The listing builds one solid part. Answer for the finished solid, in the listing's coordinates (mm). Face numbers are marked on the shaded views. A direction names the side the tool comes from. Give positions to 0.01 mm unless a question says otherwise; leave off trailing zeros. Loops run counter-clockwise (first coordinate to the right, second up) from the corner with the lowest first, then second, coordinate; pieces in that order, holes last. Notation, with made-up numbers: (33, 57) - (48, 57) arc R23 ccw to (48, 65) - close; hole circle Ø11 at (-17, -3). An arc over 180 degrees is marked (long way). Write item = value, one per line. Start each with the question number.
1) The part is cut by section C-C on y = 8. Write down the section's boundary in (x, z).
2) The part is cut by section A-A on z = 8. Write down the section's boundary in (x, y), plus the area to 3 significant figures.
3) The part is cut by section B-B on y = -45. Write down the section's boundary in (x, z), plus the area to 3 significant figures.
4) Which of the six approach directions +Z, -Z, +X, -X, +Y, -Y give full straight-line access (tool end or side, diameter ignored) to the marked faces 1, 2, 3 and 4?
5) The part is cut by section D-D on x = -38. Write down the section's boundary in (y, z), plus the area to 3 significant figures.
6) Consider probe 1 along Z at (x, y) = (-15.5, -44.5); probe 2 along Z at (x, y) = (45, 41); probe 3 along Y at (x, z) = (-13.5, 32). Determine where each line is inside the solid, lowest interval first.
7) The mould has two halves that part along X. Classify the marked faces 5, 6 and 7: +X half, -X half, draft (parallel to the pull), parting line (faces both ways), or undercut.
8) Flat-ended cylindrical pins translate along their axes: P1, Ø20, axis at x = 0.5, y = -57, coming from the -Z side; P2, Ø10, axis at x = 31.5, z = 48, coming from the +Y side; P3, Ø21, axis at x = -64.95, y = 37.5, coming from the -Z side; P4, Ø19, axis at x = 45, y = -44.5, coming from the +Z side. Find the tip coordinate at first contact, or state that the pin passes through.
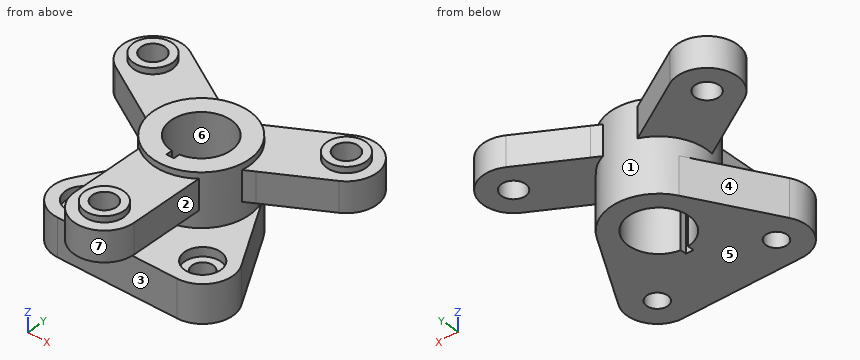
from build123d import *

# Parameters (mm, degrees)
BASE_BLOCK_DEPTH            = 25
HUB_SKETCH_64_R             = 32
HUB_64_DEPTH                = 31
THREE_START                 = -20
THREE_ARMS_120DEG_DEPTH     = 20
HUB_COLLAR_SKETCH_64_R      = 32
HUB_COLLAR_64X4_DEPTH       = 4
BOLT_BOSSES_SKETCH_3X_13_R  = 13
BOLT_BOSSES_3X_13_DEPTH     = 4
BOLT_HOLES_SKETCH_3X_8_R    = 8
BOLT_HOLES_3X_8_DEPTH       = 25
KEYED_BORE_24_DEPTH         = 80
COUNTERBORE_SKETCH_2X_12_R  = 12
COUNTERBORES_2X_12X6_DEPTH  = 6
THROUGH_HOLES_SKETCH_2X_7_R = 7
THROUGH_HOLES_2X_7_DEPTH    = 50


with BuildPart() as part:
    # Base Block Sketch → Base Block (new body)
    with BuildSketch(Plane.XY):
        with BuildLine():
            Line((-57.296551724, -34.95862069), (-27.674482759, 16.066206897))
            ThreePointArc((-27.674482759, 16.066206897), (0, 32), (27.674482759, 16.066206897))
            Line((27.674482759, 16.066206897), (57.296551724, -34.95862069))
            ThreePointArc((57.296551724, -34.95862069), (57.332449137, -54.979288897), (40, -65))
            Line((40, -65), (-40, -65))
            ThreePointArc((-40, -65), (-57.332449137, -54.979288897), (-57.296551724, -34.95862069))
        make_face()
    extrude(amount=BASE_BLOCK_DEPTH)

    # Hub Sketch _64 → Hub _64 (add)
    with BuildSketch(Plane.XY.offset(25)):
        with Locations(Location((0, 0, 0), (0, 0, 149.863023681))):
            Circle(HUB_SKETCH_64_R)
    extrude(amount=HUB_64_DEPTH)

    # Three Arms Sketch → Three Arms 120deg (add)
    with BuildSketch(Plane.XY.offset(56).offset(THREE_START)):
        with BuildLine():
            Line((-20, -75), (-20, -24.979991994))
            ThreePointArc((-20, -24.979991994), (0, -32), (20, -24.979991994))
            Line((20, -24.979991994), (20, -75))
            ThreePointArc((20, -75), (0, -95), (-20, -75))
        make_face()
        with BuildLine():
            Line((-11.633307653, 29.810504072), (-54.951905284, 54.820508076))
            ThreePointArc((-54.951905284, 54.820508076), (-82.27241336, 47.5), (-74.951905284, 20.179491924))
            Line((-74.951905284, 20.179491924), (-31.633307653, -4.830512079))
            ThreePointArc((-31.633307653, -4.830512079), (-27.712812921, 16), (-11.633307653, 29.810504072))
        make_face()
        with BuildLine():
            Line((17.280738855, 33.071049997), (54.951905284, 54.820508076))
            ThreePointArc((54.951905284, 54.820508076), (82.27146994, 47.501633873), (74.955172941, 20.181378918))
            Line((74.955172941, 20.181378918), (37.758368932, -1.303564067))
            Line((37.758368932, -1.303564067), (31.631479851, -4.842466563))
            ThreePointArc((31.631479851, -4.842466563), (27.715835779, 15.994763115), (11.633307653, 29.810504072))
            Line((11.633307653, 29.810504072), (17.280738855, 33.071049997))
        make_face()
    extrude(amount=THREE_ARMS_120DEG_DEPTH)

    # Hub Collar Sketch _64 → Hub Collar _64x4 (add)
    with BuildSketch(Plane.XY.offset(56)):
        with Locations(Location((0, 0, 0), (0, 0, 149.863023681))):
            Circle(HUB_COLLAR_SKETCH_64_R)
    extrude(amount=HUB_COLLAR_64X4_DEPTH)

    # Bolt Bosses Sketch 3x_13 → Bolt Bosses 3x_13 (add)
    with BuildSketch(Plane.XY.offset(56)):
        with Locations((-64.951905284, 37.5)):
            Circle(BOLT_BOSSES_SKETCH_3X_13_R)
        with Locations((64.951905284, 37.5)):
            Circle(BOLT_BOSSES_SKETCH_3X_13_R)
        with Locations((0, -75)):
            Circle(BOLT_BOSSES_SKETCH_3X_13_R)
    extrude(amount=BOLT_BOSSES_3X_13_DEPTH)

    # Bolt Holes Sketch 3x_8 → Bolt Holes 3x_8 (cut)
    with BuildSketch(Plane.XY.offset(60)):
        with Locations((-64.951905284, 37.5)):
            Circle(BOLT_HOLES_SKETCH_3X_8_R)
        with Locations((64.951905284, 37.5)):
            Circle(BOLT_HOLES_SKETCH_3X_8_R)
        with Locations((0, -75)):
            Circle(BOLT_HOLES_SKETCH_3X_8_R)
    extrude(amount=-BOLT_HOLES_3X_8_DEPTH, mode=Mode.SUBTRACT)

    # Keyed Bore Sketch _24 → Keyed Bore _24 (cut)
    with BuildSketch(Plane.XY.offset(60)):
        with BuildLine():
            Line((2.5, -24), (-2.5, -24))
            Line((-2.5, -24), (-2.5, -19.843134833))
            ThreePointArc((-2.5, -19.843134833), (0, 20), (2.5, -19.843134833))
            Line((2.5, -19.843134833), (2.5, -24))
        make_face()
    extrude(amount=-KEYED_BORE_24_DEPTH, mode=Mode.SUBTRACT)

    # Counterbore Sketch 2x_12 → Counterbores 2x_12x6 (cut)
    with BuildSketch(Plane.XY.offset(25)):
        with Locations((-40, -45)):
            Circle(COUNTERBORE_SKETCH_2X_12_R)
        with Locations((40, -45)):
            Circle(COUNTERBORE_SKETCH_2X_12_R)
    extrude(amount=-COUNTERBORES_2X_12X6_DEPTH, mode=Mode.SUBTRACT)

    # Through Holes Sketch 2x_7 → Through Holes 2x_7 (cut)
    with BuildSketch(Plane.XY.offset(19)):
        with Locations((-40, -45)):
            Circle(THROUGH_HOLES_SKETCH_2X_7_R)
        with Locations((40, -45)):
            Circle(THROUGH_HOLES_SKETCH_2X_7_R)
    extrude(amount=-THROUGH_HOLES_2X_7_DEPTH, mode=Mode.SUBTRACT)


solid = part.part
Answer below:
q1.outline = (-53.86, 36) - (-30.98, 36) - (-30.98, 25) - (-32.36, 25) - (-32.36, 0) - (-18.33, 0) - (-18.33, 60) - (-30.98, 60) - (-30.98, 56) - (-53.86, 56) - close; (18.33, 0) - (32.36, 0) - (32.36, 25) - (30.98, 25) - (30.98, 36) - (53.87, 36) - (53.87, 56) - (30.98, 56) - (30.98, 60) - (18.33, 60) - close
q2.outline = (-57.3, -34.96) arc R20 ccw to (-40, -65) - (40, -65) arc R20 ccw to (57.3, -34.96) - (27.67, 16.07) arc R32 ccw to (-27.67, 16.07) - close; hole circle Ø14 at (-40, -45); hole (-2.5, -24) - (2.5, -24) - (2.5, -19.84) arc R20 ccw (long way) to (-2.5, -19.84) - close; hole circle Ø14 at (40, -45)
q2.area = 6,790 mm2
q3.outline = (-60, 0) - (-47, 0) - (-47, 19) - (-52, 19) - (-52, 25) - (-60, 25) - close; (-33, 0) - (33, 0) - (33, 19) - (28, 19) - (28, 25) - (-28, 25) - (-28, 19) - (-33, 19) - close; (-20, 36) - (20, 36) - (20, 56) - (-20, 56) - close; (47, 0) - (60, 0) - (60, 25) - (52, 25) - (52, 19) - (47, 19) - close
q3.area = 2,980 mm2
q4.face_1 = none
q4.face_2 = +Z, +X, -Y
q4.face_3 = -Z, +X, -X, -Y
q4.face_4 = -Z, -X, +Y
q5.outline = (-65, 0) - (-51.71, 0) - (-51.71, 19) - (-56.83, 19) - (-56.83, 25) - (-65, 25) - close; (-38.29, 0) - (-1.72, 0) - (-1.72, 25) - (-33.17, 25) - (-33.17, 19) - (-38.29, 19) - close; (-1.15, 36) - (45.03, 36) - (45.03, 56) - (-1.15, 56) - close
q5.area = 2,110 mm2
q6.probe_1 = 0 to 25, 36 to 56
q6.probe_2 = 36 to 56
q6.probe_3 = -29.01 to -14.76, 14.76 to 29.01
q7.face_5 = draft
q7.face_6 = undercut
q7.face_7 = parting line
q8.P1 = 0
q8.P2 = 44.17
q8.P3 = 36
q8.P4 = 25
